Could you check a few things on this drawing? It's one solid part, dimensions in mm from its lowest x, y, z. A direction names the side the tool comes from. Give positions to 0.01 mm unless a question says otherwise; leave off trailing zeros. Loops run counter-clockwise (first coordinate to the right, second up) from the corner with the lowest first, then second, coordinate; pieces in that order, holes last. Notation, with made-up numbers: M 10.5,4 L 58.5,4 A18 ccw 58.5,31 Z; hole C 17,-35 d8. An arc over 180 degrees is marked long. Answer in a Markdown table with one row per item. Add a question column.
1. I'm going to push flat-ended pins straight in: pin 1 Ø4.5 at (x, y) = (15, 8.5) entering from +Z; pin 2 Ø8 at (x, z) = (21, 8.5) entering from -Y; pin 3 Ø8 at (x, y) = (63.05, 7.5) entering from -Z; pin 4 Ø1 at (y, z) = (12.5, 20) entering from -X. Where does each tip first touch, or does it pass through?
2. If we section it at B-B on y = 7.5: Count the separate pieces of the cut face and the enclosed holes in it, then the cut area to 3 significant figures.
3. If we section it at A-A on x = 63.05: List the corners of the cut face in (y, z) for me.
4. Which directions (+Z, -Z, +X, -X, +Y, -Y) give clear straight access to the entire face, cutting with the end or side of a thin tool? Please do the marked faces 1, 2 and 3.
5. If we section it at C-C on x = 5: List the corners of the cut face in (y, z) for me.
6. I need wall thicknesses on line 1 along Y through (x, z) = (63, 44); line 2 along X through (y, z) = (7.5, 2) (1 decimal); line 3 along Y through (x, z) = (25, 1). Which ranges of each line are inside material? Lowest first, please. Write a range as from..to.
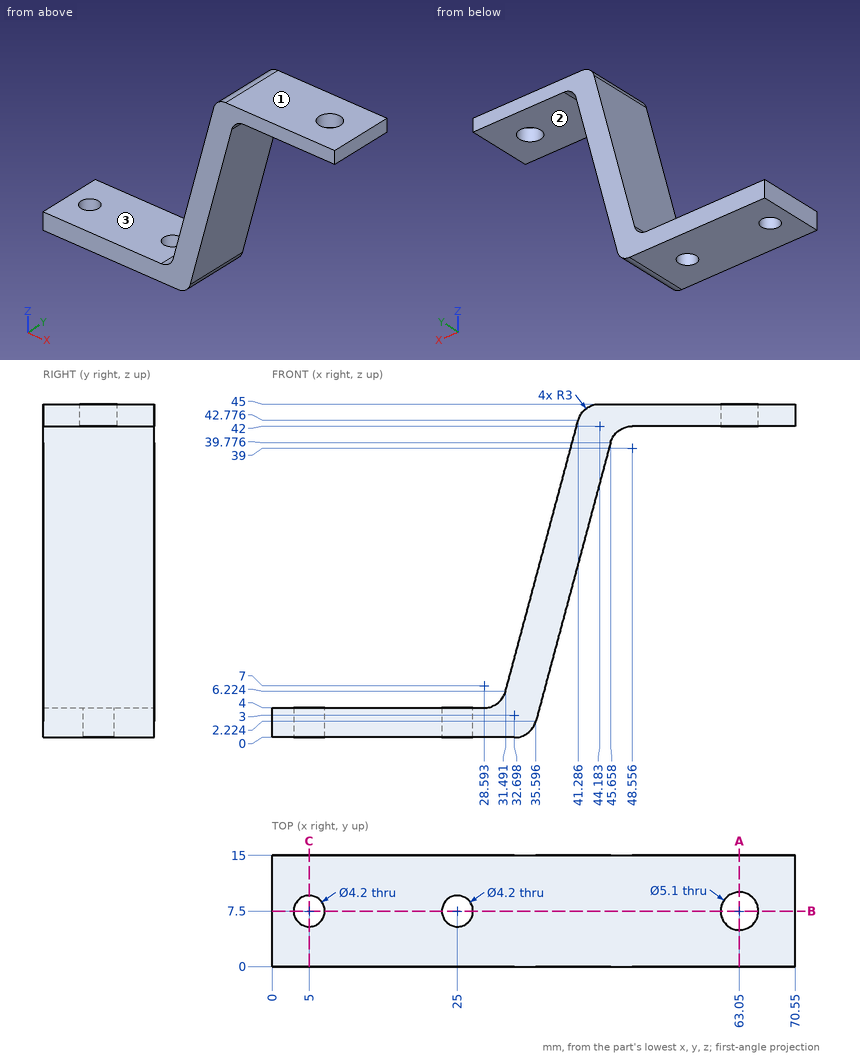
Results:
| question | item | result |
|---|---|---|
| 1 | pin 1 | z = 4 |
| 1 | pin 2 | through |
| 1 | pin 3 | z = 42 |
| 1 | pin 4 | x = 35.05 |
| 2 | separate pieces | 4 |
| 2 | enclosed holes | 0 |
| 2 | area | 377 mm2 |
| 3 | outline | M 0,42 L 4.95,42 L 4.95,45 L 0,45 Z; M 10.05,42 L 15,42 L 15,45 L 10.05,45 Z |
| 4 | face 1 | +Z, +X, -X, +Y, -Y |
| 4 | face 2 | -Z, +X, +Y, -Y |
| 4 | face 3 | +Z, -X, +Y, -Y |
| 5 | outline | M 0,0 L 5.4,0 L 5.4,4 L 0,4 Z; M 9.6,0 L 15,0 L 15,4 L 9.6,4 Z |
| 6 | line 1 | 0..4.95, 10.05..15 |
| 6 | line 2 | 0..2.9, 7.1..22.9, 27.1..35.5 |
| 6 | line 3 | 0..5.4, 9.6..15 |
